Source: CAD feature listing. Evaluate the final solid. Frame: model axes, mm. Give positions to 0.01 mm unless a question says otherwise; leave off trailing zeros. Loops run counter-clockwise (first coordinate to the right, second up) from the corner with the lowest first, then second, coordinate; pieces in that order, holes last.
from build123d import *

# Parameters (mm, degrees)
BOSS_EXTRUDE1_DEPTH          = 14
FILLET1_R                    = 10
F_10_5_10_5_DIAMETER_HOLE1_D = 10.5
F_10_5_10_5_DIAMETER_HOLE2_D = 10.5
CUT_EXTRUDE1_DEPTH           = 257.507309837
SKETCH8_W                    = 4.462850671
SKETCH8_H                    = 15.00402921
CUT_EXTRUDE2_DEPTH           = 255.008682508


with BuildPart() as part:
    # Sketch1 → Boss-Extrude1 (new body)
    with BuildSketch(Plane(origin=(0, 0, 0), x_dir=(1, 0, 0), z_dir=(0, 1, 0))):
        Polygon((0, -100), (0, 100), (80, 100), (160, 100), (160, -100), (80, -100), align=None)
    extrude(amount=BOSS_EXTRUDE1_DEPTH)

    # Fillet1
    fillet1_edges = [part.edges().sort_by_distance(p)[0] for p in [
        (0, 7, 100),
        (0, 7, -100),
    ]]
    fillet(fillet1_edges, radius=FILLET1_R)

    # Ø10.5 (10.5) Diameter Hole1 (through all)
    with Locations(Plane(origin=(0, 14, 0), x_dir=(1, 0, 0), z_dir=(0, 1, 0))):
        with Locations((60, 70), (60, -70), (60, 0)):
            Hole(F_10_5_10_5_DIAMETER_HOLE1_D / 2)

    # Ø10.5 (10.5) Diameter Hole2 (through all)
    with Locations(Plane(origin=(0, 14, 0), x_dir=(1, 0, 0), z_dir=(0, 1, 0))):
        with Locations((15, 80), (15, -80), (15, 0)):
            Hole(F_10_5_10_5_DIAMETER_HOLE2_D / 2)

    # Sketch7 → Cut-Extrude1 (cut, through all)
    with BuildSketch(Plane.XY.offset(100)):
        Polygon((149.434543456, 0), (160, 22.657694676), (160, 0), align=None)
    extrude(amount=-CUT_EXTRUDE1_DEPTH, mode=Mode.SUBTRACT)

    # Sketch8 → Cut-Extrude2 (cut, through all)
    with BuildSketch(Plane.XY.offset(100)):
        with Locations((153.731425336, 6.497985395)):
            Rectangle(SKETCH8_W, SKETCH8_H)
    extrude(amount=-CUT_EXTRUDE2_DEPTH, mode=Mode.SUBTRACT)


solid = part.part
1) Pull-direction query (X, two-part tool) for faces 1 (the cylindrical face through (2.85, 7.1, -96.99)), 2 (the flat face through (80, 7, 100)), 3 (the cylindrical face through (20.245, 6.902, -80.231)), 4 (the flat face through (151.5, 9, 1)); classes: released by +X, released by -X, zero draft, split by the parting line, or undercut.
Checks:
face 1: released by -X
face 2: zero draft
face 3: undercut
face 4: released by +X
2) Contact query for flat-ended pins moving along their axis: P1, Ø9.5, axis at x = 15, z = 0, coming from the +Y side; P2, Ø1, axis at y = 1.5, z = -39, coming from the +X side. Output: stop coordinate, or through.
Checks:
P1: passes through
P2: stops at x = 150.37
3) Ray query, probe 1 along Z at (x, y) = (15, 7); probe 2 along Z at (x, y) = (60, 9.25); probe 3 along X at (y, z) = (8.5, 76). Return the intervals inside material, ascending.
Checks:
probe 1: z = -100 to -85.25, -74.75 to -5.25, 5.25 to 74.75, 85.25 to 100
probe 2: z = -100 to -75.25, -64.75 to -5.25, 5.25 to 64.75, 75.25 to 100
probe 3: x = 0 to 11.6, 18.4 to 151.5
4) Cut plane A-A (z = 80). Return loops of the section in (x, y), and give its area (3 significant figures).
Checks:
outline: (0, 0) - (9.75, 0) - (9.75, 14) - (0, 14) - close; (20.25, 0) - (149.43, 0) - (151.5, 4.43) - (151.5, 14) - (20.25, 14) - close
area: 1,970 mm2
5) Cut plane C-C (x = 60). Return loops of the section in (y, z).
Checks:
outline: (0, -100) - (14, -100) - (14, -75.25) - (0, -75.25) - close; (0, -64.75) - (14, -64.75) - (14, -5.25) - (0, -5.25) - close; (0, 5.25) - (14, 5.25) - (14, 64.75) - (0, 64.75) - close; (0, 75.25) - (14, 75.25) - (14, 100) - (0, 100) - close
6) Cut plane B-B (y = 8.25). Return loops of the section in (x, z).
Checks:
outline: (0, -90) arc R10 ccw to (10, -100) - (151.5, -100) - (151.5, 100) - (10, 100) arc R10 ccw to (0, 90) - close; hole circle Ø10.5 at (15, -80); hole circle Ø10.5 at (15, 0); hole circle Ø10.5 at (15, 80); hole circle Ø10.5 at (60, -70); hole circle Ø10.5 at (60, 0); hole circle Ø10.5 at (60, 70)
